from build123d import *

# Parameters (mm, degrees)
SKETCH_1_W           = 35
SKETCH_1_H           = 22
EXTRUDE_1_DEPTH      = 45
SKETCH_2_W           = 35
SKETCH_2_H           = 21
CUT_EXTRUDE_1_DEPTH  = 17.5
SKETCH_3_W           = 40
SKETCH_3_H           = 8.5
CUT_EXTRUDE_2_DEPTH  = 62.10646447
FILLET_1_R           = 1.5
SKETCH_4_W           = 35
SKETCH_4_H           = 2
EXTRUDE_2_DEPTH      = 4
SKETCH_5_W           = 35
SKETCH_5_H           = 2
EXTRUDE_3_DEPTH      = 4
SKETCH_9_R           = 1.498982583
SKETCH_9_R_2         = 1.378471611
CUT_EXTRUDE_5_DEPTH  = 15
SKETCH_10_W          = 30
SKETCH_10_H          = 1.5
CUT_EXTRUDE_6_DEPTH  = 5
SKETCH_13_W          = 6
SKETCH_13_H          = 12.5
CUT_EXTRUDE_9_DEPTH  = 10
CUT_EXTRUDE_10_DEPTH = 62.854668377


with BuildPart() as part:
    # 草图1 → 拉伸1 (new body)
    with BuildSketch(Plane.XY):
        with Locations((17.5, 11)):
            Rectangle(SKETCH_1_W, SKETCH_1_H)
    extrude(amount=EXTRUDE_1_DEPTH)

    # 草图2 → 切除-拉伸1 (cut)
    with BuildSketch(Plane(origin=(20, 22, 0), x_dir=(0, 0, 1), z_dir=(0, -1, 0))):
        with Locations((22.5, 2.5)):
            Rectangle(SKETCH_2_W, SKETCH_2_H)
    extrude(amount=CUT_EXTRUDE_1_DEPTH, mode=Mode.SUBTRACT)

    # 草图3 → 切除-拉伸2 (cut, through all)
    with BuildSketch(Plane.ZY):
        with Locations((22.5, 17.75)):
            Rectangle(SKETCH_3_W, SKETCH_3_H)
    extrude(amount=-CUT_EXTRUDE_2_DEPTH, mode=Mode.SUBTRACT)

    # 圆角1
    fillet_1_edges = [part.edges().sort_by_distance(p)[0] for p in [
        (7, 9, 5),
        (28, 9, 5),
        (28, 9, 40),
        (7, 9, 40),
    ]]
    fillet(fillet_1_edges, radius=FILLET_1_R)

    # 草图4 → 拉伸2 (add)
    with BuildSketch(Plane.XY.offset(45)):
        with Locations((17.5, 23)):
            Rectangle(SKETCH_4_W, SKETCH_4_H)
    extrude(amount=-EXTRUDE_2_DEPTH)

    # 草图5 → 拉伸3 (add)
    with BuildSketch(Plane(origin=(0, 0, 0), x_dir=(-1, 0, 0), z_dir=(0, 0, -1))):
        with Locations((-17.5, 23)):
            Rectangle(SKETCH_5_W, SKETCH_5_H)
    extrude(amount=-EXTRUDE_3_DEPTH)

    # 草图9 → 切除-拉伸5 (cut)
    with BuildSketch(Plane(origin=(0, 13.5, 0), x_dir=(1, 0, 0), z_dir=(0, 1, 0))):
        with Locations(Location((3.5, -5.5, 0), (0, 0, 270))):
            Circle(SKETCH_9_R)
        with Locations(Location((3.5, -39.5, 0), (0, 0, 270))):
            Circle(SKETCH_9_R_2)
    extrude(amount=-CUT_EXTRUDE_5_DEPTH, mode=Mode.SUBTRACT)

    # 草图10 → 切除-拉伸6 (cut)
    with BuildSketch(Plane.XZ.offset(-24)):
        with Locations((15, 41.75)):
            Rectangle(SKETCH_10_W, SKETCH_10_H)
    cut_extrude_6 = extrude(amount=CUT_EXTRUDE_6_DEPTH, mode=Mode.SUBTRACT)

    # 镜向1: 切除-拉伸6 across plane
    add(cut_extrude_6.mirror(Plane(origin=(0, 0, 22.5), x_dir=(1, 0, 0), z_dir=(0, 0, -1))), mode=Mode.SUBTRACT)

    # 草图13 → 切除-拉伸9 (cut)
    with BuildSketch(Plane.XZ):
        with Locations((13, 22.5)):
            Rectangle(SKETCH_13_W, SKETCH_13_H)
    extrude(amount=-CUT_EXTRUDE_9_DEPTH, mode=Mode.SUBTRACT)

    # 草图15 → 切除-拉伸10 (cut, through all)
    with BuildSketch(Plane(origin=(35, 0, 0), x_dir=(0, 0, -1), z_dir=(1, 0, 0))):
        Polygon((-31.280717968, 11.54), (-31.35, 11.5), (-33.65, 11.5), (-33.664101615, 11.508141571), (-34.814101615, 13.5), (-30.14911144, 13.5), align=None)
    cut_extrude_10 = extrude(amount=-CUT_EXTRUDE_10_DEPTH, mode=Mode.SUBTRACT)

    # 镜向2: 切除-拉伸10 across plane
    add(cut_extrude_10.mirror(Plane(origin=(0, 0, 22.5), x_dir=(1, 0, 0), z_dir=(0, 0, -1))), mode=Mode.SUBTRACT)


solid = part.part
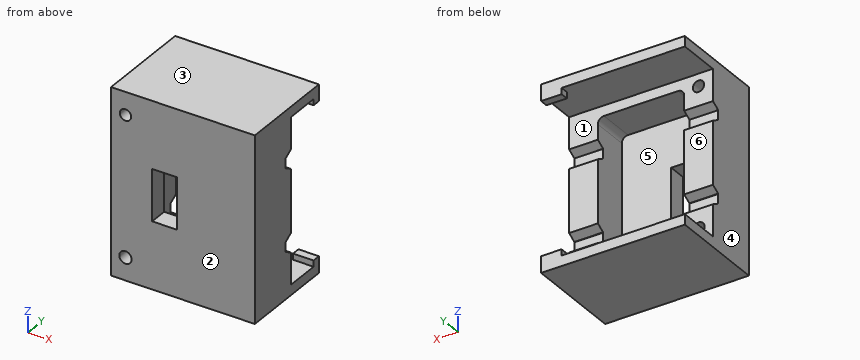
Verification items for the finished model (mm, model axes). Face numbers are marked on the shaded views. A direction names the side the tool comes from. Give positions to 0.01 mm unless a question says otherwise; leave off trailing zeros. Order: outer loops, then holes, each group sorted by start corner. A loop starts at its lowest first (then second) coordinate and runs counter-clockwise, first axis right, second up. Notation, with made-up numbers: M 71.5,74.25 L 107.5,74.25 A13 ccw 107.5,83.25 Z; hole C -9,-21.5 d4. An arc over 180 degrees is marked long. Answer as a JSON object with one key per item and string values. Group by question number.
1) Cross-section at A-A (x = 3.5). Give the number of separate pieces and of enclosed holes in the cut face, then the cut area to 3 significant figures.
2) Depth check by flat-ended pin: pin 1 Ø1.8 at (x, z) = (3.5, 32) entering from +Y; pin 2 Ø2.5 at (x, z) = (30, 32) entering from +Y; pin 3 Ø3 at (x, z) = (17, 37) entering from +Y. Enter the tip coordinate at first touch or a pass-through.
3) Access from +Z, -Z, +X, -X, +Y, -Y to the whole of each face (thin tool, end or side, straight path). Record for the marked faces 4, 5 and 6.
4) Cross-section at D-D (x = 14). Enter the section's corners in (y, z), then the cut area to 3 significant figures.
5) Cross-section at C-C (y = 5.75). Enter the section's corners in (x, z), then the cut area to 3 significant figures.
6) Mould release check, pull along Z, two halves, no side actions. Record for the marked faces 1, 2 and 3: released by +Z, released by -Z, zero draft, split by the parting line, or undercut.
7) Cross-section at B-B (z = 42). Enter the section's corners in (x, y), then the cut area to 4 significant figures.
8) Scan lines: line 1 along X through (y, z) = (9, 5.5); line 2 along Z through (x, y) = (30, 14.5); line 3 along X through (y, z) = (6.75, 18). Record each from-to range of solid material in increasing order. Write a range as [from, to].
Result sheet:
{
 "1": {"separate pieces": "3", "enclosed holes": "0", "area": "568 mm2"},
 "2": {"pin 1": "stops at y = 11.85", "pin 2": "stops at y = 12.46", "pin 3": "stops at y = 4.5"},
 "3": {"face 4": "+Z, -Z, -X, +Y, -Y", "face 5": "+Y", "face 6": "+X, -X, +Y"},
 "4": {"outline": "M 0,0 L 24,0 L 24,2.5 L 13.5,2.5 L 13.5,5 L 4.5,5 L 4.5,16.25 L 0,16.25 Z; M 0,28.75 L 4.5,28.75 L 4.5,40 L 13.5,40 L 13.5,42.5 L 24,42.5 L 24,45 L 0,45 Z", "area": "289 mm2"},
 "5": {"outline": "M 0,0 L 35,0 L 35,45 L 0,45 Z; hole C 3.5,5.5 d3; hole C 3.5,39.5 d2.76; hole M 7,6.5 A1.5 ccw 8.5,5 L 26.5,5 A1.5 ccw 28,6.5 L 28,38.5 A1.5 ccw 26.5,40 L 8.5,40 A1.5 ccw 7,38.5 Z", "area": "829 mm2"},
 "6": {"face 1": "undercut", "face 2": "zero draft", "face 3": "released by +Z"},
 "7": {"outline": "M 0,0 L 35,0 L 35,13.5 L 0,13.5 Z; M 30,22 L 35,22 L 35,24 L 30,24 Z", "area": "482.5 mm2"},
 "8": {"line 1": "x = [0, 2], [5, 7.38], [27.62, 35]", "line 2": "z = [0, 2.5], [42.5, 45]", "line 3": "x = [0, 7], [28, 35]"}
}
